from build123d import *

# Parameters (mm, degrees)
BACK_PLATE_DEPTH          = 9
TOP_ARM_DEPTH             = 12
TOP_ARM_SLOT_DEPTH        = 21
BASE_FOOT_DEPTH           = 12
MOUNTING_HOLES_SKETCH_R   = 4
MOUNTING_HOLES_2X_8_DEPTH = 12
BEARING_BOSS_30_DEPTH     = 12
BORE_SKETCH_R             = 10
BORE_20_DEPTH             = 12


with BuildPart() as part:
    # Back Plate Sketch → Back Plate (new body)
    with BuildSketch(Plane.XY):
        with BuildLine():
            Line((0, 0), (52, 0))
            Line((52, 0), (52, 96))
            ThreePointArc((52, 96), (50.242640687, 100.242640687), (46, 102))
            Line((46, 102), (6, 102))
            ThreePointArc((6, 102), (1.757359313, 100.242640687), (0, 96))
            Line((0, 96), (0, 0))
        make_face()
    extrude(amount=BACK_PLATE_DEPTH)

    # Top Arm Sketch → Top Arm (add)
    with BuildSketch(Plane.XY.offset(9)):
        with BuildLine():
            Line((26, 74), (52, 74))
            Line((52, 74), (52, 96))
            ThreePointArc((52, 96), (50.242640687, 100.242640687), (46, 102))
            Line((46, 102), (6, 102))
            ThreePointArc((6, 102), (1.757359313, 100.242640687), (0, 96))
            Line((0, 96), (0, 74))
            Line((0, 74), (26, 74))
        make_face()
    extrude(amount=TOP_ARM_DEPTH)

    # Top Arm Slot Sketch → Top Arm Slot (cut)
    with BuildSketch(Plane.XY.offset(21)):
        with BuildLine():
            Line((26, 95), (15, 95))
            ThreePointArc((15, 95), (9, 89), (15, 83))
            Line((15, 83), (37, 83))
            ThreePointArc((37, 83), (43, 89), (37, 95))
            Line((37, 95), (26, 95))
        make_face()
    extrude(amount=-TOP_ARM_SLOT_DEPTH, mode=Mode.SUBTRACT)

    # Base Foot Sketch → Base Foot (add)
    with BuildSketch(Plane.XZ):
        with BuildLine():
            Line((0, 9), (0, 34))
            ThreePointArc((0, 34), (1.757359313, 38.242640687), (6, 40))
            Line((6, 40), (46, 40))
            ThreePointArc((46, 40), (50.242640687, 38.242640687), (52, 34))
            Line((52, 34), (52, 9))
            Line((52, 9), (52, 0))
            Line((52, 0), (0, 0))
            Line((0, 0), (0, 9))
        make_face()
    extrude(amount=-BASE_FOOT_DEPTH)

    # Mounting Holes Sketch → Mounting Holes 2xØ8 (cut)
    with BuildSketch(Plane(origin=(0, 12, 0), x_dir=(1, 0, 0), z_dir=(0, 1, 0))):
        with Locations(Location((8, -32, 0), (0, 0, 270))):
            Circle(MOUNTING_HOLES_SKETCH_R)
        with Locations(Location((44, -32, 0), (0, 0, 270))):
            Circle(MOUNTING_HOLES_SKETCH_R)
    extrude(amount=-MOUNTING_HOLES_2X_8_DEPTH, mode=Mode.SUBTRACT)

    # Bearing Boss Sketch → Bearing Boss Ø30 (add)
    with BuildSketch(Plane.XY.offset(9)):
        with BuildLine():
            Line((30, 19), (30, 12))
            Line((30, 12), (22, 12))
            Line((22, 12), (22, 19.543167705))
            ThreePointArc((22, 19.543167705), (26, 49), (30, 19.543167705))
            Line((30, 19.543167705), (30, 19))
        make_face()
    extrude(amount=BEARING_BOSS_30_DEPTH)

    # Bore Sketch → Bore Ø20 (cut)
    with BuildSketch(Plane.XY.offset(21)):
        with Locations((26, 34)):
            Circle(BORE_SKETCH_R)
    extrude(amount=-BORE_20_DEPTH, mode=Mode.SUBTRACT)


solid = part.part
Geometry check sheet. Reference: the model listing, model coordinates, mm. A direction names the side the tool comes from. Round coordinates to 2 decimals unless told otherwise and drop trailing zeros. Loops run counter-clockwise (first coordinate to the right, second up) from the corner with the lowest first, then second, coordinate; pieces in that order, holes last. Notation, with made-up numbers: (-34.5, 3.25) -> (-17.5, 3.25) arc R22 cw to (-17.5, 26.25) -> close; hole circle Ø4 at (2, 59). An arc over 180 degrees is marked (long way). Answer as a JSON object with one key per item and string values. Group by question number.
Item 1: Release check for a two-part mould opening along Y. For faces 4 (the face through (26, 12, 25)), 5 (the face through (26, 23, 21)), 6 (the face through (1.804, 100.289, 10.353)) record: pulls with the +Y half, pulls with the -Y half, needs draft (parallel to the pull), parting line crosses it, or undercut.
Item 2: Cross-section at C-C, the plane z = 7. Record the cut outline in (x, y), plus the area to 3 significant figures.
Item 3: Cross-section at D-D, the plane y = 89. Record the cut outline in (x, z), plus the area to 3 significant figures.
Item 4: Cross-section at A-A, the plane x = 26. Record the cut outline in (y, z).
Item 5: Thickness scan on line 1 along X through (y, z) = (9, 32); line 2 along Y through (x, z) = (26, 13); line 3 along Y through (x, z) = (9.5, 13). Record the ranges inside material, lowest first.
Item 6: Cross-section at B-B, the plane z = 14. Record the cut outline in (x, y).
Item 7: Set-up check for faces 1 (the face through (26, 50, 9)), 2 (the face through (26, 82, 21)), 3 (the face through (26, 74, 15)): record each of +Z, -Z, +X, -X, +Y, -Y from which the full face is reachable in a straight line by a thin tool's end or side.
Item 8: Depth check by flat-ended pin: pin 1 Ø9 at (x, z) = (44, 32) entering from +Y; pin 2 Ø9 at (x, z) = (8, 32) entering from -Y; pin 3 Ø22 at (x, y) = (27, 31.5) entering from +Z; pin 4 Ø4 at (x, y) = (17, 67) entering from +Z. Enter the tip coordinate at first touch or a pass-through.
Determined:
{
 "1": {"face 4": "undercut", "face 5": "needs draft", "face 6": "pulls with the +Y half"},
 "2": {"outline": "(0, 0) -> (52, 0) -> (52, 96) arc R6 ccw to (46, 102) -> (6, 102) arc R6 ccw to (0, 96) -> close; hole (15, 83) -> (37, 83) arc R6 ccw to (37, 95) -> (15, 95) arc R6 ccw to start", "area": "4,910 mm²"},
 "3": {"outline": "(0, 0) -> (9, 0) -> (9, 21) -> (0, 21) -> close; (43, 0) -> (52, 0) -> (52, 21) -> (43, 21) -> close", "area": "378 mm²"},
 "4": {"outline": "(0, 0) -> (83, 0) -> (83, 21) -> (74, 21) -> (74, 9) -> (49, 9) -> (49, 21) -> (44, 21) -> (44, 9) -> (24, 9) -> (24, 21) -> (12, 21) -> (12, 40) -> (0, 40) -> close; (95, 0) -> (102, 0) -> (102, 21) -> (95, 21) -> close"},
 "5": {"line 1": "x = 0 to 4, 12 to 40, 48 to 52", "line 2": "y = 0 to 24, 44 to 49, 74 to 83, 95 to 102", "line 3": "y = 0 to 12, 74 to 86.6, 91.4 to 102"},
 "6": {"outline": "(0, 0) -> (52, 0) -> (52, 12) -> (30, 12) -> (30, 19.54) arc R15 ccw (long way) to (22, 19.54) -> (22, 12) -> (0, 12) -> close; (0, 74) -> (52, 74) -> (52, 96) arc R6 ccw to (46, 102) -> (6, 102) arc R6 ccw to (0, 96) -> close; hole (15, 83) -> (37, 83) arc R6 ccw to (37, 95) -> (15, 95) arc R6 ccw to start; hole circle Ø20 at (26, 34)"},
 "7": {"face 1": "+Z", "face 2": "+Z, +X, -X, +Y", "face 3": "+Z, +X, -X"},
 "8": {"pin 1": "stops at y = 12", "pin 2": "stops at y = 0", "pin 3": "stops at z = 21", "pin 4": "stops at z = 9"}
}
